Could you check a few things on this model? Use its own coordinates, in mm. A direction names the side the tool comes from. Round coordinates to 2 decimals unless told otherwise and drop trailing zeros. Loops run counter-clockwise (first coordinate to the right, second up) from the corner with the lowest first, then second, coordinate; pieces in that order, holes last.
from build123d import *


with BuildPart() as part:
    # Sketch 181 → 旋转1 (revolve)
    with BuildSketch(Plane.XY, mode=Mode.PRIVATE) as revolve_1_sk:
        Polygon((-35, 45.965688775), (-34, 45), (34, 45), (35, 45.965688775), (35, 55), (30, 55), (30, 49.8), (28, 49.8), (28, 50), (-34, 50), (-35, 49), align=None)
    revolve(revolve_1_sk.sketch.rotate(Axis((-35, 0, 0), (1, 0, 0)), 90), axis=Axis((-35, 0, 0), (1, 0, 0)))


solid = part.part
Item 1: We'd pull the mould along Z, two halves only. Please class faces 3 (the cylindrical face through (0.476, 39.923, 20.765)), 4 (the flat face through (30, -41, -29)), 5 (the cylindrical face through (-3.43, -15.02, 47.69)): released by +Z, released by -Z, zero draft, split by the parting line, or undercut.
Results list:
face 3: undercut
face 4: zero draft
face 5: split by the parting line
Item 2: If we section it at A-A, the plane y = 0: Please give me the cut outline in (x, z), then the cut area to 3 significant figures.
Results list:
outline: (-35, -49) - (-34, -50) - (28, -50) - (28, -49.8) - (30, -49.8) - (30, -55) - (35, -55) - (35, -45.97) - (34, -45) - (-34, -45) - (-35, -45.97) - close; (-35, 45.97) - (-34, 45) - (34, 45) - (35, 45.97) - (35, 55) - (30, 55) - (30, 49.8) - (28, 49.8) - (28, 50) - (-34, 50) - (-35, 49) - close
area: 746 mm2
Item 3: For faces 1 (the cylindrical face through (28.99, 30.3, -39.52)), 2 (the flat face through (-35, 14, -44)), which set-ups out of +Z, -Z, +X, -X, +Y, -Y let a thin tool reach every point of the face, with its end or its side?
Results list:
face 1: none
face 2: +Z, -Z, -X, +Y, -Y
Item 4: If I drill on line 1 along Y through (x, z) = (-15, 0); line 2 along X through (y, z) = (24, -45.5); line 3 along Z through (x, y) = (-22, 2.5), over which ranges is the centre line in solid material (lowest first)?
Results list:
line 1: y = -50 to -45, 45 to 50
line 2: x = 30 to 35
line 3: z = -49.94 to -44.93, 44.93 to 49.94
Item 5: Will these pins go through, and if not, where does the flat tip stop? pin 1 (12 mm diameter, centred on x = -22, z = 12, fed in from -Y); pin 2 (2 mm diameter, centred on x = 16, y = -34.5, fed in from +Z); pin 3 (3 mm diameter, centred on x = 7, y = 11.5, fed in from -Z).
Results list:
pin 1: stops at y = -49.64
pin 2: stops at z = 37.12
pin 3: stops at z = -48.99
Item 6: If we section it at C-C, the plane x = 18: Please give me the cut outline in (y, z).
Results list:
outline: circle Ø100 at (0, 0); hole circle Ø90 at (0, 0)
